Geometry check sheet. Reference: the model listing, model coordinates, mm. Face numbers are marked on the shaded views. A direction names the side the tool comes from. Coordinates: 2 decimals unless noted, no trailing zeros. Order: outer loops, then holes, each group sorted by start corner. A loop starts at its lowest first (then second) coordinate and runs counter-clockwise, first axis right, second up. Notation, with made-up numbers: (81, 8) - (94, 8) arc R21 cw to (94, 35) - close; hole circle Ø7 at (4, -11.75). An arc over 180 degrees is marked (long way). Use CSV: the item, a comma, the result in double quotes. Start each with the question number.
1) Depth check by flat-ended pin: P1, Ø0.7, axis at x = 21.5, z = 0, coming from the -Y side. Enter the tip coordinate at first touch or a pass-through.
2) Thickness scan on probe 1 along Y at (x, z) = (0, -0.1); probe 2 along X at (y, z) = (-0.7, -0.6); probe 3 along Y at (x, z) = (0, 0.5). Record the ranges inside material, lowest first. Write a range as [from, to].
3) Tool access check on the marked faces 1 and 2. Record the directions out of +Z, -Z, +X, -X, +Y, -Y that give a thin tool (end or side, any length) a straight path to the whole face; none if there is none.
4) Sectioned sample at A-A, the plane x = 22. Record the cut outline in (y, z), and give its area (3 significant figures).
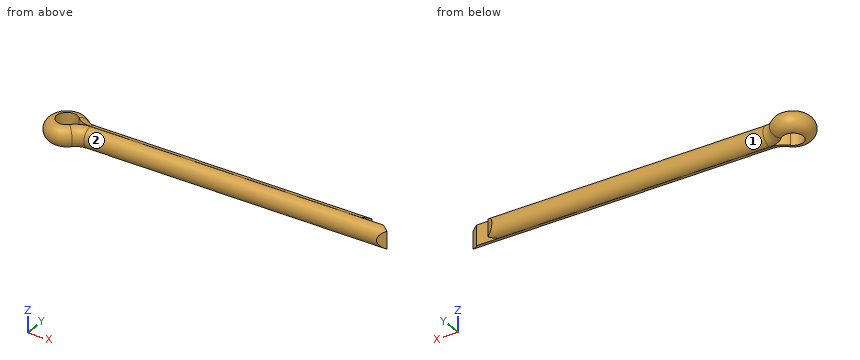
from build123d import *

# Parameters (mm, degrees)
CUT_EXTRUDE1_DEPTH      = 38.288770437
CUT_EXTRUDE1_DEPTH_BACK = 38.288770437


with BuildPart() as part:
    # Sweep2: sweep along a path in Dimension sketch
    with BuildLine(Plane.XY) as sweep2_path:
        Line((34.7, 1.15), (2.7, 1.15))
        ThreePointArc((2.7, 1.15), (2.133929691, 1.265530578), (1.658403483, 1.593642961))
        ThreePointArc((1.658403483, 1.593642961), (-2.3, 0), (1.658403483, -1.593642961))
        ThreePointArc((1.658403483, -1.593642961), (2.133929691, -1.265530578), (2.7, -1.15))
        Line((2.7, -1.15), (37.2, -1.15))
    # Sketch2 → Sweep2 (sweep)
    with BuildSketch(Plane(origin=(34.7, 1.15, 0), x_dir=(0, 0, 1), z_dir=(-1, 0, 0))):
        with BuildLine():
            Line((-1.149956521, -1.14), (1.149956521, -1.14))
            ThreePointArc((1.149956521, -1.14), (0, 0), (-1.149956521, -1.14))
        make_face()
    sweep(path=sweep2_path.line)

    # Sketch3 → Cut-Extrude1 (cut, two sides: drawn at the far end of the back side and taken through both)
    with BuildSketch(Plane.XY.offset(-CUT_EXTRUDE1_DEPTH_BACK)):
        Polygon((34.7, 0.57), (33.882315934, 1.15), (37.21, 1.15), (37.21, -1.15), (36.375313858, -1.15), (37.2, -0.58), (36.382315934, 0), (33.875313858, 0), align=None)
    extrude(amount=CUT_EXTRUDE1_DEPTH + CUT_EXTRUDE1_DEPTH_BACK, mode=Mode.SUBTRACT)


solid = part.part
Evaluation:
1,P1,"y = -1.15"
2,probe 1,"[-2.3, -1.16], [1.16, 2.3]"
2,probe 2,"[-2.01, -0.92], [0.94, 37.03]"
2,probe 3,"[-2.19, -1.16], [1.16, 2.19]"
3,face 1,"+X, +Y"
3,face 2,"+X, -Y"
4,outline,"(-0.01, -1.15) - (-0.01, 1.15) arc R1.15 ccw to start; (0.01, -1.15) arc R1.15 ccw to (0.01, 1.15) - close"
4,area,"4.11 mm²"
